Can you work these out from the model? Positions are in its coordinate system, mm. Face numbers are marked on the shaded views. Give positions to 0.01 mm unless a question says otherwise; leave off trailing zeros. Order: outer loops, then holes, each group sorted by start corner. A loop starts at its lowest first (then second) coordinate and runs counter-clockwise, first axis right, second up. Notation, with made-up numbers: (49.25, 6) - (58.25, 6) arc R19 cw to (58.25, 36) - close; hole circle Ø7 at (22.25, -9). An arc over 180 degrees is marked (long way). Answer as CSV lines item,"result".
```python
from build123d import *

# Parameters (mm, degrees)
BASE_BAR_EXTRUDE_75MM_DEPTH    = 37.5
SKETCH1_4_W                    = 430
SKETCH1_4_H                    = 10
PROFILE_REGION_BOSS_25MM_DEPTH = 12.5
SKETCH1_5_W                    = 430
SKETCH1_5_H                    = 10
PROFILE_REGION_BOSS_45MM_DEPTH = 22.5


with BuildPart() as part:
    # Bar Profile Sketch → Base Bar Extrude 75mm (new, symmetric)
    with BuildSketch(Plane.XY):
        Polygon((0, 25), (0, 0), (430, 0), (450, 0), (450, 25), (350, 35), (282, 35), (267, 20), (127, 20), (142, 35), (100, 35), align=None)
    extrude(amount=BASE_BAR_EXTRUDE_75MM_DEPTH, both=True)

    # Sketch1_4 → Profile Region Boss 25mm (add, symmetric)
    with BuildSketch(Plane.XY):
        with Locations((215, -5)):
            Rectangle(SKETCH1_4_W, SKETCH1_4_H)
    extrude(amount=PROFILE_REGION_BOSS_25MM_DEPTH, both=True)

    # Sketch1_5 → Profile Region Boss 45mm (add, symmetric)
    with BuildSketch(Plane.XY):
        with Locations((215, -15)):
            Rectangle(SKETCH1_5_W, SKETCH1_5_H)
    extrude(amount=PROFILE_REGION_BOSS_45MM_DEPTH, both=True)


solid = part.part
```
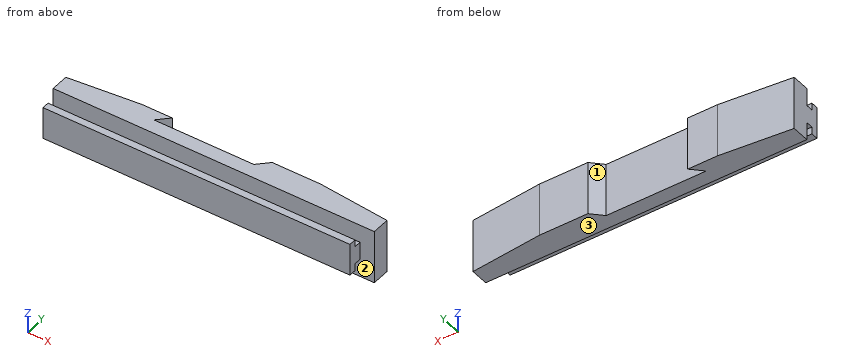
1) I want a section at D-D on z = 7.5. Write out the boundary of the cut face in (x, y), plus the area to 4 significant figures.
Answer block:
outline,"(0, -20) - (430, -20) - (430, 0) - (450, 0) - (450, 25) - (350, 35) - (282, 35) - (267, 20) - (127, 20) - (142, 35) - (100, 35) - (0, 25) - close"
area,"21,250 mm2"
2) I need wall thicknesses on line 1 along Z through (x, y) = (210, -12.5); line 2 along Z through (x, y) = (38, -3.5); line 3 along X through (y, z) = (-12, -10). Which ranges of each line are inside material? Lowest first, please. Write a range as [from, to].
Answer block:
line 1,"[-22.5, 22.5]"
line 2,"[-12.5, 12.5]"
line 3,"[0, 430]"
3) If we mould it in two halves opening along Y, with no side actions, what happens to the marked faces 1, 2 and 3? For each: +Y half, -Y half, draft (parallel to the pull), parting line (faces both ways), or undercut.
Answer block:
face 1,"+Y half"
face 2,"undercut"
face 3,"draft"
4) I'm going to push flat-ended pins straight in: P1, Ø5, axis at x = 220, y = -15.5, coming from the +Z side; P2, Ø5, axis at x = 254, y = -12.5, coming from the -Z side; P3, Ø11, axis at x = 167.5, z = -16.5, coming from the +Y side. Where does each tip first touch, or does it pass through?
Answer block:
P1,"z = 22.5"
P2,"z = -22.5"
P3,"y = 20"
5) I want a section at A-A on z = -17. Write out the boundary of the cut face in (x, y), plus the area to 4 significant figures.
Answer block:
outline,"(0, -20) - (430, -20) - (430, -10) - (0, -10) - close; (0, 0) - (450, 0) - (450, 25) - (350, 35) - (282, 35) - (267, 20) - (127, 20) - (142, 35) - (100, 35) - (0, 25) - close"
area,"16,950 mm2"
6) I want a section at C-C on x = 359.5. Write out the boundary of the cut face in (y, z), plus the area to 3 significant figures.
Answer block:
outline,"(-20, -22.5) - (-10, -22.5) - (-10, -12.5) - (0, -12.5) - (0, -37.5) - (34.05, -37.5) - (34.05, 37.5) - (0, 37.5) - (0, 12.5) - (-10, 12.5) - (-10, 22.5) - (-20, 22.5) - close"
area,"3,250 mm2"
7) I want a section at B-B on x = 137.5. Write out the boundary of the cut face in (y, z).
Answer block:
outline,"(-20, -22.5) - (-10, -22.5) - (-10, -12.5) - (0, -12.5) - (0, -37.5) - (20, -37.5) - (20, 37.5) - (0, 37.5) - (0, 12.5) - (-10, 12.5) - (-10, 22.5) - (-20, 22.5) - close; (30.5, -37.5) - (35, -37.5) - (35, 37.5) - (30.5, 37.5) - close"
